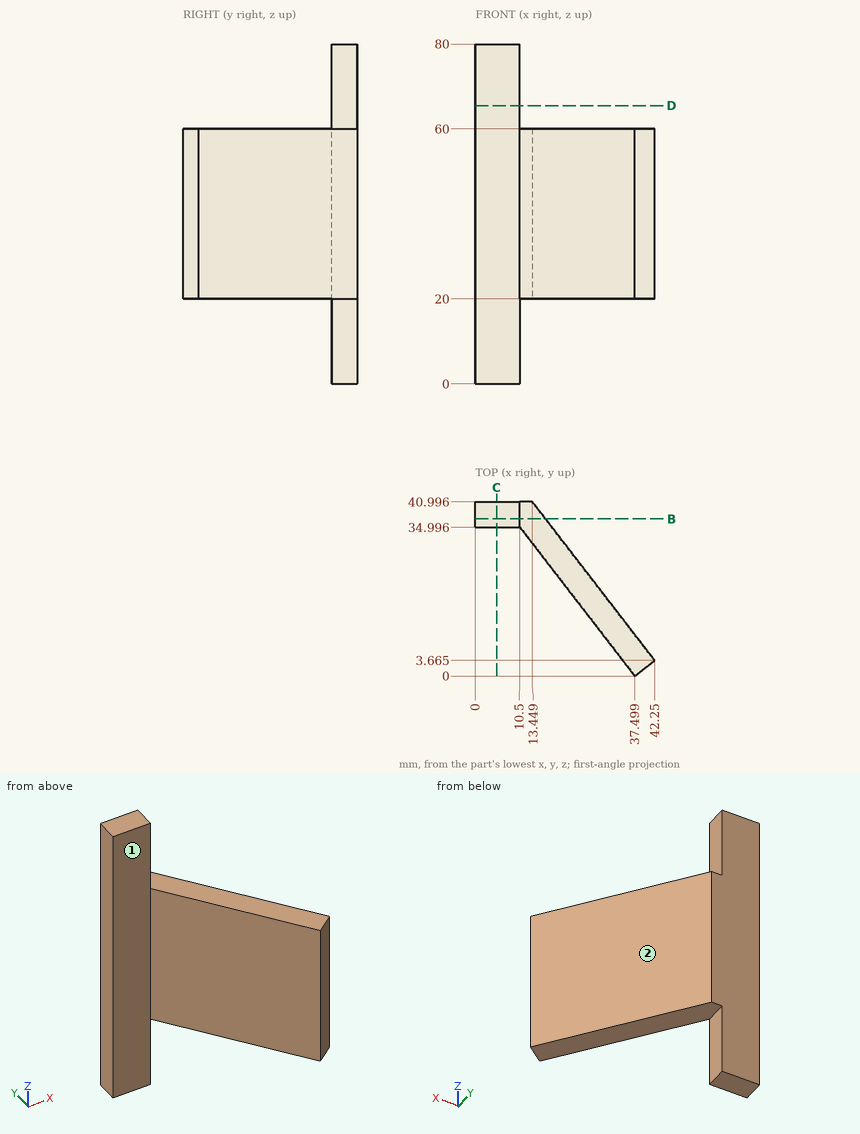
Source: three-view drawing plus pictorial views. Frame: mm from the lowest corner of the part. A direction names the side the tool comes from. Coordinates: 2 decimals unless noted, no trailing zeros. Order: outer loops, then holes, each group sorted by start corner. A loop starts at its lowest first (then second) coordinate and runs counter-clockwise, first axis right, second up.
1) Section B-B (y = 37). Return loops of the section in (x, z).
Result sheet:
outline: (0, 0) - (10.5, 0) - (10.5, 20) - (16.53, 20) - (16.53, 60) - (10.5, 60) - (10.5, 80) - (0, 80) - close
2) Section C-C (x = 5). Return loops of the section in (y, z) (1 decimal).
Result sheet:
outline: (35, 0) - (41, 0) - (41, 80) - (35, 80) - close
3) Ray query, probe 1 along Z at (x, y) = (36, 4.5); probe 2 along Y at (x, z) = (7, 6.5) (1 decimal); probe 3 along X at (y, z) = (36, 68). Return the intervals inside material, ascending.
Result sheet:
probe 1: z = 20 to 60
probe 2: y = 35 to 41
probe 3: x = 0 to 10.5
4) Set-up query: the marked faces 1 and 2. Return all of +Z, -Z, +X, -X, +Y, -Y with unobstructed straight access to the full face (end or side cutting, diameter ignored); none if empty.
Result sheet:
face 1: +Z, -Z, -X, -Y
face 2: +Z, -Z, +X, +Y
5) First-contact query: P1, Ø4, axis at x = 34.5, z = 29.5, coming from the +Y side; P2, Ø6, axis at y = 14.5, z = 16, coming from the -X side; P3, Ø16, axis at x = 31, y = 19, coming from the -Z side; P4, Ø6.5, axis at y = 37.5, z = 69, coming from the +X side. Flat tips, straight axial feed; report the tip coordinate or a pass-through.
Result sheet:
P1: stops at y = 16.3
P2: passes through
P3: stops at z = 20
P4: stops at x = 10.5
6) Section D-D (z = 65.5). Return loops of the section in (x, y) (1 decimal).
Result sheet:
outline: (0, 35) - (10.5, 35) - (10.5, 41) - (0, 41) - close
